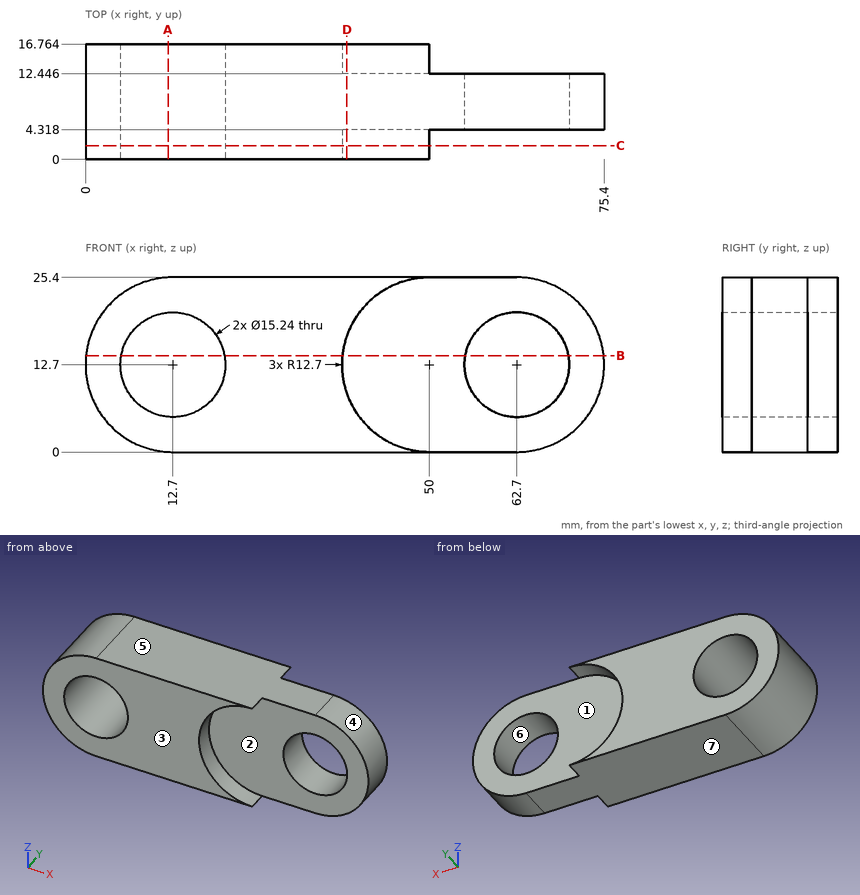
Study the drawing (mm; zero at the part's minimum x, y, z) and answer. A direction names the side the tool comes from. Give positions to 0.01 mm unless a question says otherwise; leave off trailing zeros. Loops run counter-clockwise (first coordinate to the right, second up) from the corner with the lowest first, then second, coordinate; pieces in that order, holes last. Notation, with made-up numbers: (57, 70) - (110, 70) arc R12 ccw to (110, 90) - close; hole circle Ø9 at (73.5, -38). An arc over 180 degrees is marked (long way). Answer as CSV lines item,"result". Start each with the question number.
1) Find section A-A (x = 12). Write down the section's boundary in (y, z).
2) Straight lines are drawn through the part: L1, parallel to X at y = 7, z = 12.7; L2, parallel to Z at x = 62.7, y = 9.5; L3, parallel to X at y = 5, z = 18.5. For each, find the intervals that lie inside material, in ascending order. Write a range as from..to.
3) Each of these flat-tipped pins is pushed along its axis until it touches: pin 1 Ø10 at (x, z) = (43, 14.5) entering from -Y; pin 2 Ø7.5 at (x, z) = (56.5, 11) entering from +Y; pin 3 Ø8 at (y, z) = (12.5, 4.5) entering from -X; pin 4 Ø5 at (x, z) = (17, 13.5) entering from +Y. Where does it stop, or does it pass through?
4) Which of the six approach directions +Z, -Z, +X, -X, +Y, -Y give full straight-line access (tool end or side, diameter ignored) to the marked faces 1, 2 and 3?
5) Find section C-C (y = 2). Write down the section's boundary in (x, z), then the cut area to 3 significant figures.
6) Find section B-B (z = 14). Write down the section's boundary in (x, y).
7) Find section D-D (x = 38). Write down the section's boundary in (y, z), then the cut area to 3 significant figures.
8) Determine the mould class of the marked faces 4, 5, 6 and 7 for opening direction Z: released by +Z, released by -Z, zero draft, split by the parting line, or undercut.
Findings below:
1,outline,"(0, 0.02) - (16.76, 0.02) - (16.76, 5.11) - (0, 5.11) - close; (0, 20.29) - (16.76, 20.29) - (16.76, 25.38) - (0, 25.38) - close"
2,L1,"0..5.08, 20.32..55.08, 70.32..75.4"
2,L2,"0..5.08, 20.32..25.4"
2,L3,"1.4..7.76, 17.64..57.76, 67.64..74"
3,pin 1,"y = 4.32"
3,pin 2,"y = 12.45"
3,pin 3,"x = 0.71"
3,pin 4,"through"
4,face 1,"+X, +Y"
4,face 2,"+X, -Y"
4,face 3,"+Z, -Z, +X, -X, -Y"
5,outline,"(12.7, 0) - (50, 0) arc R12.7 cw to (50, 25.4) - (12.7, 25.4) arc R12.7 ccw to start; hole circle Ø15.24 at (12.7, 12.7)"
5,area,"765 mm^2"
6,outline,"(0.07, 0) - (5.19, 0) - (5.19, 16.76) - (0.07, 16.76) - close; (20.21, 0) - (37.37, 0) - (37.37, 4.32) - (55.19, 4.32) - (55.19, 12.45) - (37.37, 12.45) - (37.37, 16.76) - (20.21, 16.76) - close; (70.21, 4.32) - (75.33, 4.32) - (75.33, 12.45) - (70.21, 12.45) - close"
7,outline,"(0, 0) - (16.76, 0) - (16.76, 8.54) - (12.45, 8.54) - (12.45, 16.86) - (16.76, 16.86) - (16.76, 25.4) - (0, 25.4) - (0, 16.86) - (4.32, 16.86) - (4.32, 8.54) - (0, 8.54) - close"
7,area,"354 mm^2"
8,face 4,"split by the parting line"
8,face 5,"released by +Z"
8,face 6,"undercut"
8,face 7,"released by -Z"
